from build123d import *

# Parameters (mm, degrees)
BOSS_EXTRUDE1_DEPTH = 28


with BuildPart() as part:
    # Sketch1 → Boss-Extrude1 (new body)
    with BuildSketch(Plane(origin=(0, 0, 0), x_dir=(1, 0, 0), z_dir=(0, 1, 0))):
        Polygon((2011.523887052, 1584.007884982), (2396.523887052, 1584.007884982), (2411.523887052, 1599.007884982), (2411.523887052, 1644.007884982), (2011.523887052, 1604.007884982), align=None)
    extrude(amount=BOSS_EXTRUDE1_DEPTH)


solid = part.part
Design review of the part built by this model. Coordinates are the model's own, in mm. Round coordinates to 2 decimals unless told otherwise and drop trailing zeros. Loops run counter-clockwise (first coordinate to the right, second up) from the corner with the lowest first, then second, coordinate; pieces in that order, holes last. Notation, with made-up numbers: M 84,88.25 L 120,88.25 A29 ccw 120,116.25 Z; hole C -8,-2 d10. An arc over 180 degrees is marked long. Answer as a JSON object with one key per item and string values.
Item 1: Wall thickness on L1, parallel to Z at x = 2270, y = 8.5; L2, parallel to X at y = 20.25, z = -1598; L3, parallel to Z at x = 2200.5, y = 24: over which ranges is each line inside the solid? List them lowest first. Write a range as from..to.
Answer sheet:
{"L1": "z = -1629.86..-1584.01", "L2": "x = 2011.52..2410.52", "L3": "z = -1622.91..-1584.01"}
Item 2: We need section B-B on z = -1610. Give the boundary of the cut face in (x, y).
Answer sheet:
{"outline": "M 2071.45,0 L 2411.52,0 L 2411.52,28 L 2071.45,28 Z"}
Item 3: Clearance check with flat-ended pins moving along their axes: P1, Ø10, axis at x = 2103.5, y = 4, coming from the -Z side; P2, Ø2, axis at x = 2249.5, y = 24.5, coming from the -Z side; P3, Ø6, axis at x = 2227, z = -1629.5, coming from the +Y side (3 decimals). State where each tip first meets the part, or that it passes through.
Answer sheet:
{"P1": "stops at z = -1613.71", "P2": "stops at z = -1627.91", "P3": "passes through"}
Item 4: We need section A-A on y = 7.75. Give the boundary of the cut face in (x, z).
Answer sheet:
{"outline": "M 2011.52,-1604.01 L 2411.52,-1644.01 L 2411.52,-1599.01 L 2396.52,-1584.01 L 2011.52,-1584.01 Z"}
Item 5: We need section C-C on x = 2289. Give the boundary of the cut face in (y, z).
Answer sheet:
{"outline": "M 0,-1631.76 L 28,-1631.76 L 28,-1584.01 L 0,-1584.01 Z"}
